from build123d import *

# Parameters (mm, degrees)
SKETCH_1_W          = 25.5
SKETCH_1_H          = 40
EXTRUDE_1_DEPTH     = 6.5
SKETCH_2_R          = 6
EXTRUDE_2_DEPTH     = 40
SKETCH_3_W          = 13.5
SKETCH_3_H          = 7.5
CUT_EXTRUDE_1_DEPTH = 30.925950277
SKETCH_5_R          = 3.5
CUT_EXTRUDE_2_DEPTH = 29.174678348
CHAMFER_1_SIZE      = 3


with BuildPart() as part:
    # 草图1 → 凸台-拉伸1 (new body)
    with BuildSketch(Plane(origin=(0, 0, 0), x_dir=(1, 0, 0), z_dir=(0, 1, 0))):
        Rectangle(SKETCH_1_W, SKETCH_1_H)
    extrude(amount=EXTRUDE_1_DEPTH)

    # 草图2 → 凸台-拉伸2 (add)
    with BuildSketch(Plane.XY.offset(20)):
        with Locations((12.75, 6)):
            Circle(SKETCH_2_R)
    extrude(amount=-EXTRUDE_2_DEPTH)

    # 草图3 → 切除-拉伸1 (cut, through all)
    with BuildSketch(Plane.XZ):
        with Locations((12, 16.25)):
            Rectangle(SKETCH_3_W, SKETCH_3_H)
        with Locations((12, -16.25)):
            Rectangle(SKETCH_3_W, SKETCH_3_H)
    extrude(amount=-CUT_EXTRUDE_1_DEPTH, mode=Mode.SUBTRACT)

    # 草图5 → 切除-拉伸2 (cut, through all)
    with BuildSketch(Plane(origin=(0, 6.5, 0), x_dir=(1, 0, 0), z_dir=(0, 1, 0))):
        with Locations(Location((-2.239565186, 12, 0), (0, 0, 270))):
            Circle(SKETCH_5_R)
        with Locations(Location((-2.239565186, -12, 0), (0, 0, 270))):
            Circle(SKETCH_5_R)
    extrude(amount=-CUT_EXTRUDE_2_DEPTH, mode=Mode.SUBTRACT)

    # 倒角1
    chamfer_1_edges = [part.edges().sort_by_distance(p)[0] for p in [
        (-2.239565186, 6.5, -15.5),
        (-2.239565186, 6.5, 8.5),
    ]]
    chamfer(chamfer_1_edges, length=CHAMFER_1_SIZE)


solid = part.part
Source: CAD feature listing. Evaluate the final solid. Frame: model axes, mm. A direction names the side the tool comes from. Round coordinates to 2 decimals unless told otherwise and drop trailing zeros. Loops run counter-clockwise (first coordinate to the right, second up) from the corner with the lowest first, then second, coordinate; pieces in that order, holes last. Notation, with made-up numbers: (44.5, 5.5) - (72.5, 5.5) arc R26 ccw to (72.5, 36.5) - close; hole circle Ø6 at (-6.75, -24.75). An arc over 180 degrees is marked (long way). Write item = value, one per line. Start each with the question number.
(1) Pin query (flat end, axial travel): pin 1 (5 mm diameter, centred on x = 9.5, y = 8.5, fed in from +Z); pin 2 (5 mm diameter, centred on y = 8.5, z = 15.5, fed in from -X); pin 3 (10 mm diameter, centred on x = -5, z = -2, fed in from +Y); pin 4 (3 mm diameter, centred on y = 10, z = 13, fed in from +X). Return the tip coordinate at first contact, or that it passes through.
(2) Pull-direction query (Z, two-part tool) for faces 1 (the face through (-5, 6.5, 0)), 2 (the face through (-2.086, 1.774, -15.497)), 3 (the face through (-4, 3, -20)); classes: +Z half, -Z half, draft (parallel to the pull), parting line (faces both ways), or undercut.
(3) Section query D-D, the plane y = 1.75. Output: boundary loops of the cut face in (x, z), plus the area to 3 significant figures.
(4) Set-up query: faces 4 (the face through (5.25, 3, 16)), 5 (the face through (12, 6, -12.5)), 6 (the face through (-4, 3, 20)). Return all of +Z, -Z, +X, -X, +Y, -Y with unobstructed straight access to the full face (end or side cutting, diameter ignored); none if empty.
(5) Section query C-C, the plane x = -1. State how many separate pieces and enclosed holes the cut face has, plus the area to 3 significant figures.
(6) Ray query, line 1 along Z through (x, y) = (-4, 1.25); line 2 along Y through (x, z) = (-2, -1.5); line 3 along Z through (x, y) = (10, 10.5). Return the intervals inside material, ascending. Write a range as from..to.
(7) Section query B-B, the plane y = 4.25. Output: boundary loops of the cut face in (x, z), plus the area to 3 significant figures.
(8) Section query A-A, the plane z = -12. Output: boundary loops of the cut face in (x, y).
Conclusion:
q1.pin_1 = 12.5
q1.pin_2 = -12.75
q1.pin_3 = 6.5
q1.pin_4 = 18.16
q2.face_1 = draft
q2.face_2 = undercut
q2.face_3 = -Z half
q3.outline = (-12.75, -20) - (5.25, -20) - (5.25, -12.5) - (16.99, -12.5) - (16.99, 12.5) - (5.25, 12.5) - (5.25, 20) - (-12.75, 20) - close; hole circle Ø7 at (-2.24, -12); hole circle Ø7 at (-2.24, 12)
q3.area = 936 mm2
q4.face_4 = +Z, +X, +Y, -Y
q4.face_5 = -Z, +X, +Y, -Y
q4.face_6 = +Z, +X, -X, +Y, -Y
q5.separate_pieces = 3
q5.enclosed_holes = 0
q5.area = 156 mm2
q6.line_1 = -20..-15.03, -8.97..8.97, 15.03..20
q6.line_2 = 0..6.5
q6.line_3 = -12.5..12.5
q7.outline = (-12.75, -20) - (5.25, -20) - (5.25, -12.5) - (18.49, -12.5) - (18.49, 12.5) - (5.25, 12.5) - (5.25, 20) - (-12.75, 20) - close; hole circle Ø8.5 at (-2.24, -12); hole circle Ø8.5 at (-2.24, 12)
q7.area = 937 mm2
q8.outline = (-12.75, 0) - (-5.74, 0) - (-5.74, 3.5) - (-8.74, 6.5) - (-12.75, 6.5) - close; (1.26, 0) - (12.75, 0) arc R6 ccw (long way) to (6.77, 6.5) - (4.26, 6.5) - (1.26, 3.5) - close
